The figure shows three views and two pictorial views of one solid part (mm, origin at its lowest corner). Answer the questions. A direction names the side the tool comes from. Give positions to 0.01 mm unless a question says otherwise; leave off trailing zeros. Loops run counter-clockwise (first coordinate to the right, second up) from the corner with the lowest first, then second, coordinate; pieces in that order, holes last. Notation, with made-up numbers: (36.5, 21) - (80.5, 21) arc R25 ccw to (80.5, 49) - close; hole circle Ø10 at (14, 45). An arc over 180 degrees is marked (long way). Write item = value, one per line.
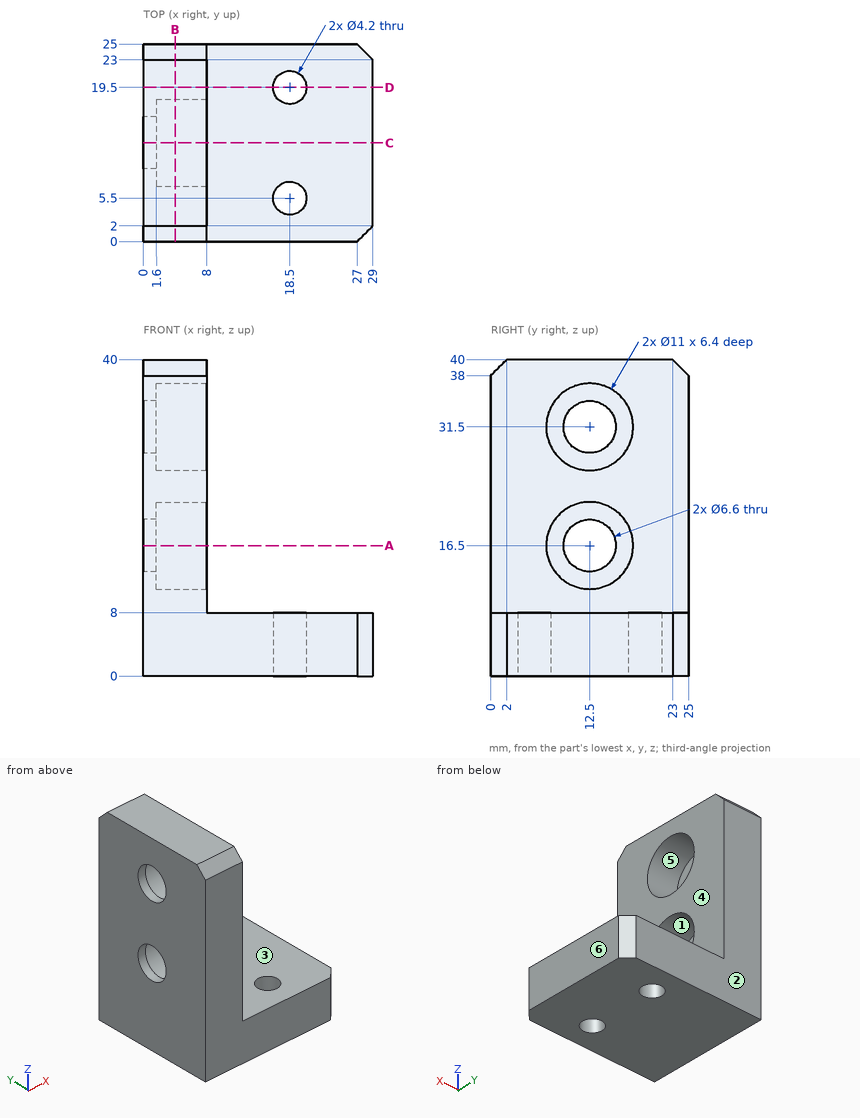
1) A cutting plane is placed at B-B on x = 4. Determine the outline of the cut face in (y, z).
Output:
outline = (0, 0) - (25, 0) - (25, 38) - (23, 40) - (2, 40) - (0, 38) - close; hole circle Ø11 at (12.5, 16.5); hole circle Ø11 at (12.5, 31.5)
2) A cutting plane is placed at C-C on y = 12.5. Determine the outline of the cut face in (x, z).
Output:
outline = (0, 0) - (29, 0) - (29, 8) - (8, 8) - (8, 11) - (1.6, 11) - (1.6, 13.2) - (0, 13.2) - close; (0, 19.8) - (1.6, 19.8) - (1.6, 22) - (8, 22) - (8, 26) - (1.6, 26) - (1.6, 28.2) - (0, 28.2) - close; (0, 34.8) - (1.6, 34.8) - (1.6, 37) - (8, 37) - (8, 40) - (0, 40) - close
3) A cutting plane is placed at A-A on z = 16.5. Determine the outline of the cut face in (x, y).
Output:
outline = (0, 0) - (8, 0) - (8, 7) - (1.6, 7) - (1.6, 9.2) - (0, 9.2) - close; (0, 15.8) - (1.6, 15.8) - (1.6, 18) - (8, 18) - (8, 25) - (0, 25) - close
4) Find the intervals of material crossed by probe 1 along Z at (x, y) = (5.5, 12.25); probe 2 along Y at (x, z) = (5.75, 31.5); probe 3 along Y at (x, z) = (0.7, 31.5), in increasing order.
Output:
probe_1 = 0 to 11.01, 21.99 to 26.01, 36.99 to 40
probe_2 = 0 to 7, 18 to 25
probe_3 = 0 to 9.2, 15.8 to 25
5) A cutting plane is placed at D-D on y = 19.5. Determine the outline of the cut face in (x, z), then the cut area to 3 significant figures.
Output:
outline = (0, 0) - (16.4, 0) - (16.4, 8) - (8, 8) - (8, 40) - (0, 40) - close; (20.6, 0) - (29, 0) - (29, 8) - (20.6, 8) - close
area = 454 mm²
6) Each of these flat-tipped pins is pushed along its axis until it touches: P1, Ø7.5, axis at y = 12.5, z = 16.5, coming from the -X side; P2, Ø3, axis at y = 2.5, z = 29.5, coming from the +X side; P3, Ø6, axis at y = 12.5, z = 31.5, coming from the -X side; P4, Ø3.5, axis at y = 10.5, z = 29.5, coming from the +X side. Where does it stop, or does it pass through?
Output:
P1 = 0
P2 = 8
P3 = through
P4 = 1.6
7) The mould has two halves that part along Y. Classify the marked faces 1, 2 and 3: pulls with the +Y half, pulls with the -Y half, needs draft (parallel to the pull), parting line crosses it, or undercut.
Output:
face_1 = undercut
face_2 = pulls with the +Y half
face_3 = needs draft
8) A tool of negligible diameter and unlimited length cuts with its end or side. For the marked faces 4, 5 and 6, from which of +Z, -Z, +X, -X, +Y, -Y can it reach the whole face along a straight path? Write none if from no direction.
Output:
face_4 = +Z, +X, +Y, -Y
face_5 = +X
face_6 = +Z, -Z, +X, +Y, -Y
